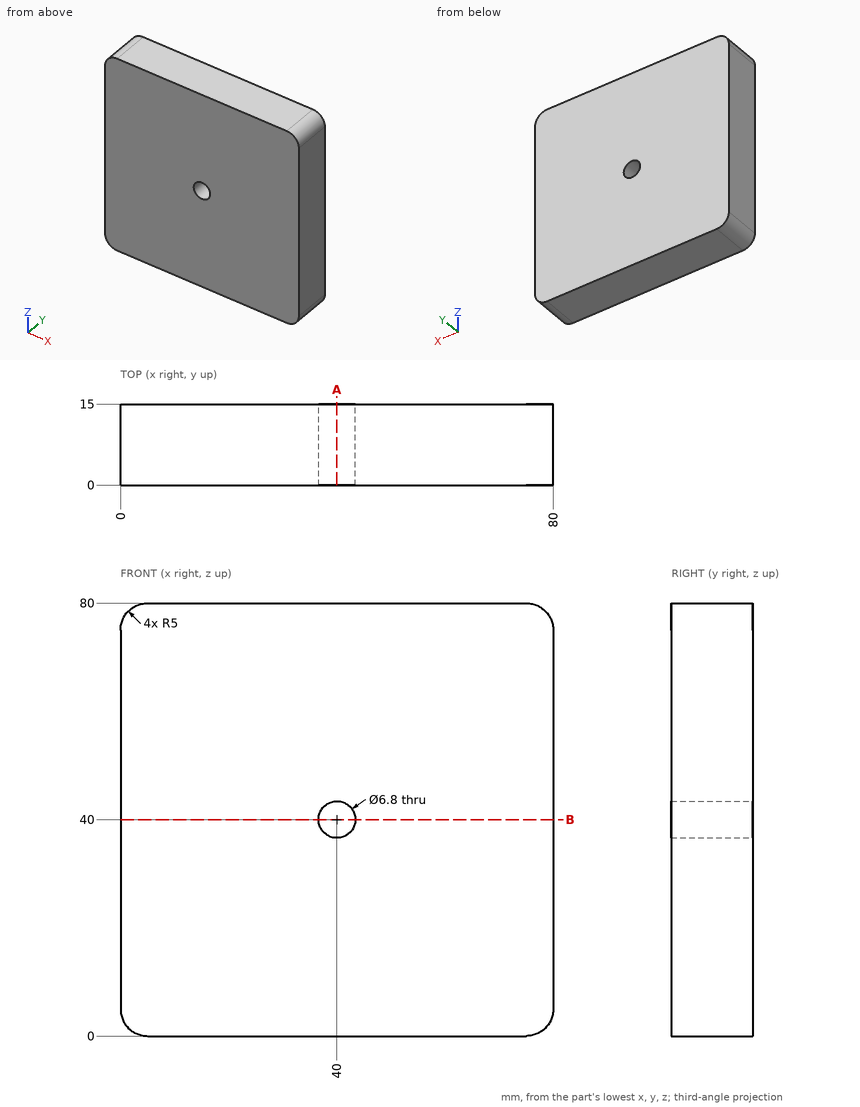
Geometry: see drawing. Coordinates: mm, zero at the bounding-box minimum. Give positions to 0.01 mm unless a question says otherwise; leave off trailing zeros. Loops run counter-clockwise (first coordinate to the right, second up) from the corner with the lowest first, then second, coordinate; pieces in that order, holes last. Notation, with made-up numbers: (-17, -34.5) - (41, -34.5) arc R25 ccw to (41, 1.5) - close; hole circle Ø7 at (-21.5, -14.5). An arc over 180 degrees is marked (long way). Use CSV: the item, a comma, the result in double quotes.
1) Cut plane B-B (z = 40). Output: boundary loops of the cut face in (x, y), and give its area (3 significant figures).
Worked out:
outline,"(0, 0) - (36.6, 0) - (36.6, 15) - (0, 15) - close; (43.4, 0) - (80, 0) - (80, 15) - (43.4, 15) - close"
area,"1,100 mm^2"
2) Line query: line 1 (Z direction, x = 40, y = 5.75); line 2 (X direction, y = 8, z = 42). Output: solid intervals per line, ascending.
Worked out:
line 1,"z = 0 to 36.6, 43.4 to 80"
line 2,"x = 0 to 37.25, 42.75 to 80"
3) Cut plane A-A (x = 40). Output: boundary loops of the cut face in (y, z), and give its area (3 significant figures).
Worked out:
outline,"(0, 0) - (15, 0) - (15, 36.6) - (0, 36.6) - close; (0, 43.4) - (15, 43.4) - (15, 80) - (0, 80) - close"
area,"1,100 mm^2"
